Input: part model. Units: mm. Frame: model coordinates. A direction names the side the tool comes from. Give positions to 0.01 mm unless a question says otherwise; leave off trailing zeros. Answer as a JSON object with one key per item and string values. Group by question number.
```python
from build123d import *

# Parameters (mm, degrees)
SKETCH_1_W             = 136
SKETCH_1_H             = 100
EXTRUDE_1_DEPTH        = 20
HOLE_WIZARD_M8_1_D     = 6.8
HOLE_WIZARD_M8_1_DEPTH = 19.75
HOLE_WIZARD_M8_1_TIP   = 2.042926105
HOLE_WIZARD_M8_2_D     = 6.8
HOLE_WIZARD_M8_2_DEPTH = 19.75
HOLE_WIZARD_M8_2_TIP   = 2.042926105


with BuildPart() as part:
    # 草图1 → 凸台-拉伸1 (new body)
    with BuildSketch(Plane(origin=(0, 0, 0), x_dir=(0, 0, -1), z_dir=(1, 0, 0))):
        Rectangle(SKETCH_1_W, SKETCH_1_H)
    extrude(amount=EXTRUDE_1_DEPTH)

    # M8 螺纹孔1
    with Locations(Plane(origin=(0, 50, 0), x_dir=(1, 0, 0), z_dir=(0, 1, 0))):
        with Locations((9.910141203, 45), (9.910141203, -45), (9.734330512, 0)):
            Hole(HOLE_WIZARD_M8_1_D / 2, depth=HOLE_WIZARD_M8_1_DEPTH)
            with Locations((0, 0, -(HOLE_WIZARD_M8_1_DEPTH + HOLE_WIZARD_M8_1_TIP / 2))):  # 118° drill point
                Cone(0, HOLE_WIZARD_M8_1_D / 2, HOLE_WIZARD_M8_1_TIP, mode=Mode.SUBTRACT)

    # M8 螺纹孔2
    with Locations(Plane(origin=(0, -50, 0), x_dir=(-1, 0, 0), z_dir=(0, -1, 0))):
        with Locations((-10, 45), (-10, 0), (-10, -45)):
            Hole(HOLE_WIZARD_M8_2_D / 2, depth=HOLE_WIZARD_M8_2_DEPTH)
            with Locations((0, 0, -(HOLE_WIZARD_M8_2_DEPTH + HOLE_WIZARD_M8_2_TIP / 2))):  # 118° drill point
                Cone(0, HOLE_WIZARD_M8_2_D / 2, HOLE_WIZARD_M8_2_TIP, mode=Mode.SUBTRACT)


solid = part.part
```
1. Material intervals for L1, parallel to X at y = 40.25, z = -45; L2, parallel to X at y = -40, z = -45, sorted ascending.
2. Mould query, pull axis X, two halves, no side actions, for faces 4 (the flat face through (5, 50, 1)), 5 (the cylindrical face through (6.594, 39.987, 1.302)), 6 (the flat face through (0, 1, 1)). Classes: pulls with the +X half, pulls with the -X half, needs draft (parallel to the pull), parting line crosses it, or undercut.
3. First-contact query: P1, Ø12, axis at y = 39, z = 33.5, coming from the -X side; P2, Ø4, axis at x = 10, z = 45, coming from the +Y side; P3, Ø4, axis at x = 10, z = -45, coming from the -Y side; P4, Ø5.5, axis at x = 10, z = 0, coming from the -Y side. Flat tips, straight axial feed; report the tip coordinate or a pass-through.
4. Reachability of faces 1 (the flat face through (10, -1, -68)), 2 (the cylindrical face through (12.416, 39.987, -47.298)), 3 (the cylindrical face through (13.14, -39.99, 1.3)) from +Z, -Z, +X, -X, +Y, -Y: full face, straight path, thin tool, end or side. Return the list, or none.
Geometry results:
{
 "1": {"L1": "0 to 6.51, 13.31 to 20", "L2": "0 to 6.6, 13.4 to 20"},
 "2": {"face 4": "needs draft", "face 5": "undercut", "face 6": "pulls with the -X half"},
 "3": {"P1": "x = 0", "P2": "y = 29.46", "P3": "y = -29.41", "P4": "y = -29.86"},
 "4": {"face 1": "-Z, +X, -X, +Y, -Y", "face 2": "+Y", "face 3": "-Y"}
}
